Geometry check sheet. Reference: drawing and pictorial views, mm from the part's lowest x, y, z. A direction names the side the tool comes from. Give positions to 0.01 mm unless a question says otherwise; leave off trailing zeros. Write each loop counter-clockwise with the first axis right and the second up, starting at its lowest first coordinate (ties: lowest second). Pieces come first, ordered by that corner, then holes. Notation, with made-up numbers: M 11,12.5 L 29,12.5 A31 cw 29,44.5 Z; hole C 11.25,84 d4. An arc over 180 degrees is marked long. One line per item, written item: value. Start each with the question number.
1. Gauge pin test, flat ends, axial feed: pin 1 (1 mm diameter, centred on x = 2.5, z = 1, fed in from +Y); pin 2 (1 mm diameter, centred on y = 6, z = 1.5, fed in from +X). Record the tip position at first contact, or that the pin passes through.
2. Tool access check on the marked faces 1 and 2. Record the directions out of +Z, -Z, +X, -X, +Y, -Y that give a thin tool (end or side, any length) a straight path to the whole face; none if there is none.
3. Cross-section at A-A on y = 2.25. Record the cut outline in (x, z), then the cut area to 3 significant figures.
4. Scan lines: line 1 (Z direction, x = 1.75, y = 6.75); line 2 (Y direction, x = 1.3, z = 2.3); line 3 (X direction, y = 6.25, z = 0.95). Record each from-to range of solid material in increasing order.
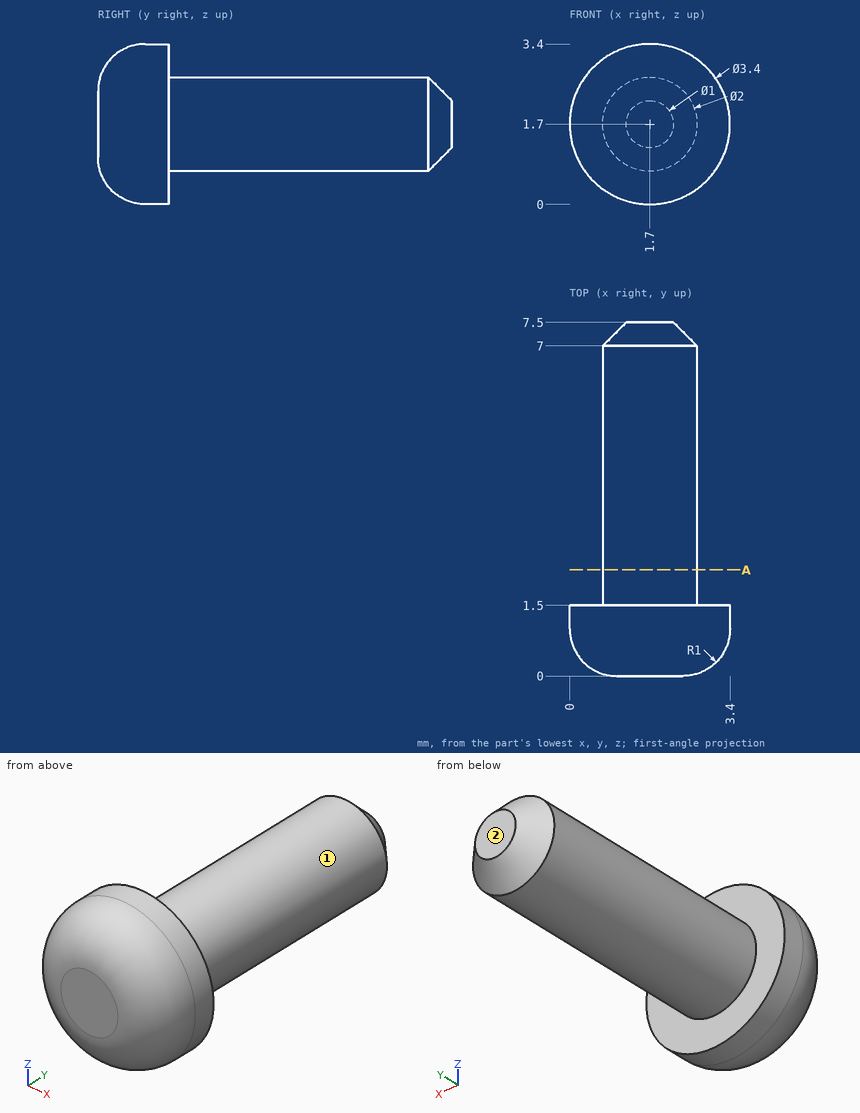
Report:
1. pin 1: stops at y = 7.44
1. pin 2: stops at x = 2.7
2. face 1: +Y
2. face 2: +Z, -Z, +X, -X, +Y
3. outline: C 1.7,1.7 d2
3. area: 3.14 mm^2
4. line 1: z = 0.7 to 2.7
4. line 2: y = 0 to 7.28
4. line 3: x = 1.04 to 2.36
